from build123d import *

# Parameters (mm, degrees)
GB_T6728_2002_60_X_60_X_4_1_DEPTH = 495
CUT_EXTRUDE_1_REACH               = 258.43
SKETCH_5_R                        = 10
CUT_EXTRUDE_2_REACH               = 258.43
SKETCH_6_R                        = 10


with BuildPart() as part:
    # Sketch1 → 冷弯空心方管gb∕t6728-2002 60 X 60 X 4(1) (new body)
    with BuildSketch(Plane.YZ.offset(-247.5)):
        with BuildLine():
            Line((-22, -30), (22, -30))
            ThreePointArc((22, -30), (27.656854249, -27.656854249), (30, -22))
            Line((30, -22), (30, 22))
            ThreePointArc((30, 22), (27.656854249, 27.656854249), (22, 30))
            Line((22, 30), (-22, 30))
            ThreePointArc((-22, 30), (-27.656854249, 27.656854249), (-30, 22))
            Line((-30, 22), (-30, -22))
            ThreePointArc((-30, -22), (-27.656854249, -27.656854249), (-22, -30))
        make_face()
        with BuildLine():
            Line((-22, -26), (22, -26))
            ThreePointArc((22, -26), (24.828427125, -24.828427125), (26, -22))
            Line((26, -22), (26, 22))
            ThreePointArc((26, 22), (24.828427125, 24.828427125), (22, 26))
            Line((22, 26), (-22, 26))
            ThreePointArc((-22, 26), (-24.828427125, 24.828427125), (-26, 22))
            Line((-26, 22), (-26, -22))
            ThreePointArc((-26, -22), (-24.828427125, -24.828427125), (-22, -26))
        make_face(mode=Mode.SUBTRACT)
    extrude(amount=GB_T6728_2002_60_X_60_X_4_1_DEPTH)

    # 切除-拉伸1: up to this face of the body (flat: up to its plane)
    cut_extrude_1_end = Plane(part.part.faces().sort_by_distance((0, 0, -30))[0])
    # 草图5 → 切除-拉伸1 (cut, up to the picked face)
    with BuildSketch(Plane.XY.offset(30), mode=Mode.PRIVATE) as cut_extrude_1_sk1:
        with Locations((-160, 0)):
            Circle(SKETCH_5_R)
    cut_extrude_1_tool1 = split(extrude(cut_extrude_1_sk1.sketch, amount=-CUT_EXTRUDE_1_REACH, mode=Mode.PRIVATE), bisect_by=cut_extrude_1_end, keep=Keep.BOTH, mode=Mode.PRIVATE)
    add(cut_extrude_1_tool1.solids().sort_by(Axis((-160, 0, 30), (0, 0, -1)))[0], mode=Mode.SUBTRACT)

    # 切除-拉伸2: up to this face of the body (flat: up to its plane)
    cut_extrude_2_end = Plane(part.part.faces().sort_by_distance((0, -30, 0))[0])
    # 草图6 → 切除-拉伸2 (cut, up to the picked face)
    with BuildSketch(Plane(origin=(0, 30, 0), x_dir=(1, 0, 0), z_dir=(0, 1, 0)), mode=Mode.PRIVATE) as cut_extrude_2_sk1:
        with Locations(Location((-160, 0, 0), (0, 0, 270))):
            Circle(SKETCH_6_R)
    cut_extrude_2_tool1 = split(extrude(cut_extrude_2_sk1.sketch, amount=-CUT_EXTRUDE_2_REACH, mode=Mode.PRIVATE), bisect_by=cut_extrude_2_end, keep=Keep.BOTH, mode=Mode.PRIVATE)
    add(cut_extrude_2_tool1.solids().sort_by(Axis((-160, 30, 0), (0, -1, 0)))[0], mode=Mode.SUBTRACT)


solid = part.part
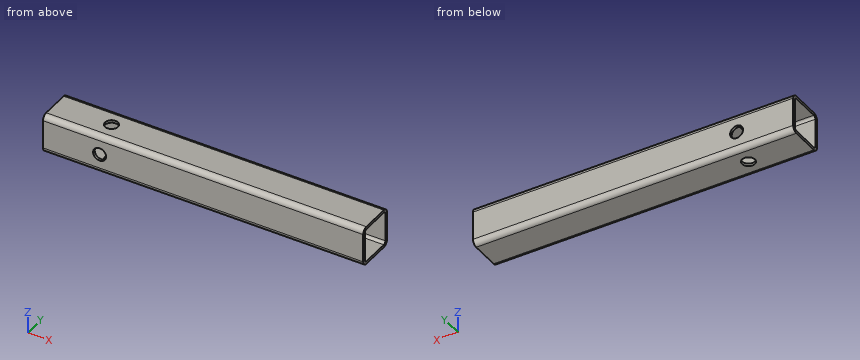
Here's how the part is built. I have some questions about the finished solid (model axes, mm). Give positions to 0.01 mm unless a question says otherwise; leave off trailing zeros. Order: outer loops, then holes, each group sorted by start corner. A loop starts at its lowest first (then second) coordinate and runs counter-clockwise, first axis right, second up. Notation, with made-up numbers: (-16, -27.5) -> (25, -27.5) arc R13 ccw to (25, -18.5) -> close; hole circle Ø4 at (-24, 17). An arc over 180 degrees is marked (long way). One line per item, written item: value. Start each with the question number.
1. Imagine slicing it at D-D, the plane x = -160. Count the separate pieces of the cut face and the enclosed holes in it, plus the area to 3 significant figures.
2. I need wall thicknesses on probe 1 along Y at (x, z) = (-216.5, 7); probe 2 along X at (y, z) = (-27, 0). Which ranges of each line are inside material? Lowest first, please. Write a range as from..to.
3. Imagine slicing it at B-B, the plane x = 179.5. List the corners of the cut face in (y, z) for me.
4. Imagine slicing it at A-A, the plane y = -17. List the corners of the cut face in (x, z) for me.
5. Imagine slicing it at C-C, the plane z = 0. List the corners of the cut face in (x, y) for me, plus the area to 3 significant figures.
Values follow:
1. separate pieces: 4
1. enclosed holes: 0
1. area: 535 mm2
2. probe 1: y = -30..-26, 26..30
2. probe 2: x = -247.5..-170, -150..247.5
3. outline: (-30, -22) arc R8 ccw to (-22, -30) -> (22, -30) arc R8 ccw to (30, -22) -> (30, 22) arc R8 ccw to (22, 30) -> (-22, 30) arc R8 ccw to (-30, 22) -> close; hole (-26, -22) arc R4 ccw to (-22, -26) -> (22, -26) arc R4 ccw to (26, -22) -> (26, 22) arc R4 ccw to (22, 26) -> (-22, 26) arc R4 ccw to (-26, 22) -> close
4. outline: (-247.5, -30) -> (247.5, -30) -> (247.5, -26) -> (-247.5, -26) -> close; (-247.5, 26) -> (247.5, 26) -> (247.5, 30) -> (-247.5, 30) -> close
5. outline: (-247.5, -30) -> (-170, -30) -> (-170, -26) -> (-247.5, -26) -> close; (-247.5, 26) -> (-170, 26) -> (-170, 30) -> (-247.5, 30) -> close; (-150, -30) -> (247.5, -30) -> (247.5, -26) -> (-150, -26) -> close; (-150, 26) -> (247.5, 26) -> (247.5, 30) -> (-150, 30) -> close
5. area: 3,800 mm2
